from build123d import *

# Parameters (mm, degrees)
SKETCH1_W           = 25
SKETCH1_H           = 25
BOSS_EXTRUDE1_DEPTH = 32
M12_TAPPED_HOLE1_D  = 10.2


with BuildPart() as part:
    # Sketch1 → Boss-Extrude1 (new body)
    with BuildSketch(Plane(origin=(0, 0, 0), x_dir=(1, 0, 0), z_dir=(0, 1, 0))):
        Rectangle(SKETCH1_W, SKETCH1_H)
    extrude(amount=BOSS_EXTRUDE1_DEPTH)

    # M12 Tapped Hole1 (through all)
    with Locations(Plane(origin=(0, 32, 0), x_dir=(1, 0, 0), z_dir=(0, 1, 0))):
        with Locations((0, 0)):
            Hole(M12_TAPPED_HOLE1_D / 2)


solid = part.part
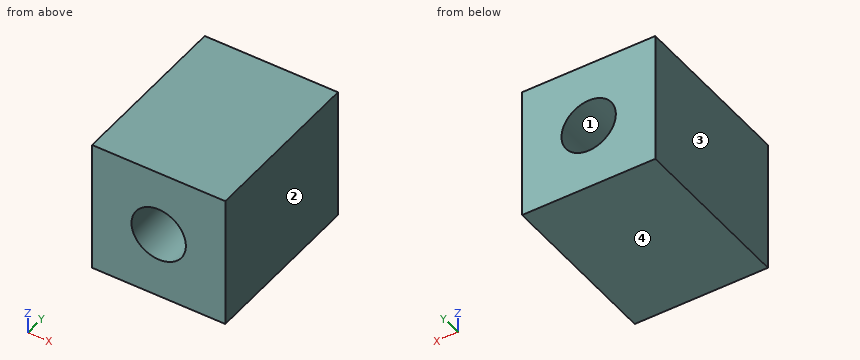
Can you work these out from the model? Positions are in its coordinate system, mm. Face numbers are marked on the shaded views. Coordinates: 2 decimals unless noted, no trailing zeros. Loops run counter-clockwise (first coordinate to the right, second up) from the corner with the lowest first, then second, coordinate; pieces in that order, holes last. Notation, with made-up numbers: M 26,9.5 L 68,9.5 A22 ccw 68,22.5 Z; hole C -25,34.25 d7. An arc over 180 degrees is marked long. Answer as CSV lines item,"result". Start each with the question number.
1. Suppose I cut it at B-B, the plane y = 29. List the corners of the cut face in (x, z) for me.
2. Thinking about a two-plate mould opening in X: for the marked faces 1, 2, 3 and 4, which applies, +X half, -X half, draft (parallel to the pull), parting line (faces both ways), or undercut?
3. Suppose I cut it at A-A, the plane x = 0. List the corners of the cut face in (y, z) for me.
4. Suppose I cut it at C-C, the plane z = 0. List the corners of the cut face in (x, y) for me.
5. If I drill on probe 1 along Z at (x, y) = (0, 24); probe 2 along Z at (x, y) = (-4, 7.5); probe 3 along X at (y, z) = (19.5, 2.75), over which ranges is the centre line in solid material (lowest first)? Write a range as [from, to].
6. For pin 1 Ø8 at (x, z) = (0, 0) entering from +Y (3 decimals), with a flat end and sliding along its axis, tell me the tip position at first contact or that it passes through.
Output:
1,outline,"M -12.5,-12.5 L 12.5,-12.5 L 12.5,12.5 L -12.5,12.5 Z; hole C 0,0 d10.2"
2,face 1,"undercut"
2,face 2,"+X half"
2,face 3,"-X half"
2,face 4,"draft"
3,outline,"M 0,-12.5 L 32,-12.5 L 32,-5.1 L 0,-5.1 Z; M 0,5.1 L 32,5.1 L 32,12.5 L 0,12.5 Z"
4,outline,"M -12.5,0 L -5.1,0 L -5.1,32 L -12.5,32 Z; M 5.1,0 L 12.5,0 L 12.5,32 L 5.1,32 Z"
5,probe 1,"z = [-12.5, -5.1], [5.1, 12.5]"
5,probe 2,"z = [-12.5, -3.16], [3.16, 12.5]"
5,probe 3,"x = [-12.5, -4.3], [4.3, 12.5]"
6,pin 1,"passes through"
